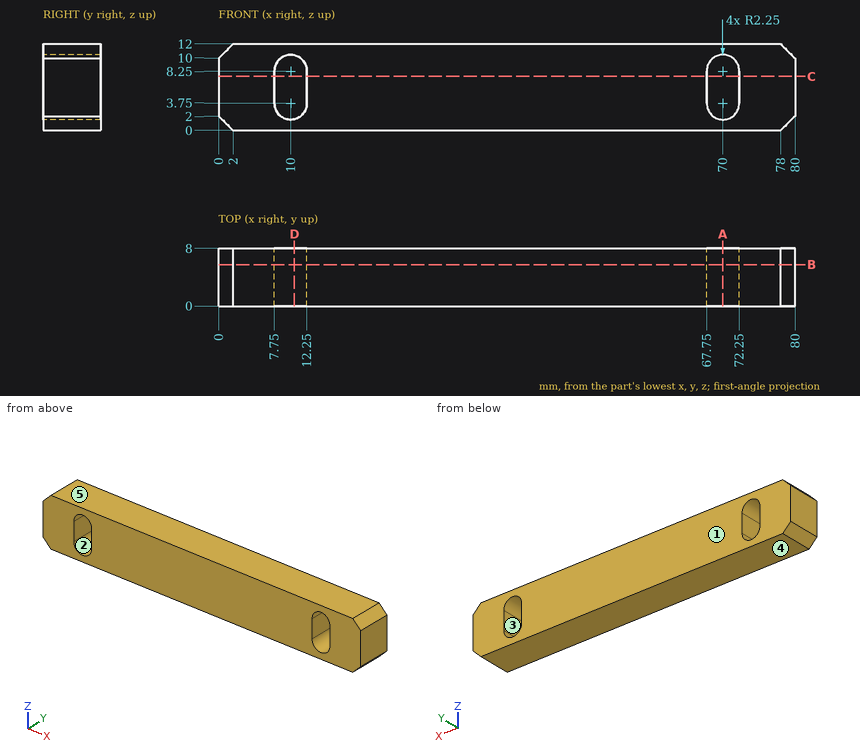
Check sheet for the drawn part. Datum: minimum x, y, z corner. Units: mm. A direction names the side the tool comes from. Round coordinates to 2 decimals unless told otherwise and drop trailing zeros. Write each loop counter-clockwise with the first axis right and the second up, starting at its lowest first coordinate (ties: lowest second). Pieces come first, ordered by that corner, then holes. Notation, with made-up numbers: (4, -15) -> (24, -15) arc R30 ccw to (24, 22) -> close; hole circle Ø8 at (21.5, 74.25). An arc over 180 degrees is marked (long way). Write each question's results on one line, items separated by ' | '. Start each with the question number.
1. Cross-section at C-C (z = 7.5). Enter the section's corners in (x, y), then the cut area to 3 significant figures.
2. Set-up check for the marked faces 1 and 2: record each of +Z, -Z, +X, -X, +Y, -Y from which the full face is reachable in a straight line by a thin tool's end or side.
3. Cross-section at D-D (x = 10.5). Enter the section's corners in (y, z).
4. Cross-section at B-B (y = 5.75). Enter the section's corners in (x, z).
5. Material ranges on probe 1 along X at (y, z) = (6.5, 6.5); probe 2 along Z at (x, y) = (69, 4.75); probe 3 along Z at (x, y) = (8.5, 6.75), recorded low to high. Write a range as from..to.
6. Cross-section at A-A (x = 70). Enter the section's corners in (y, z), then the cut area to 3 significant figures.
7. Draft check along Z on the marked faces 3, 4 and 5. Enter one of: +Z half, -Z half, draft (parallel to the pull), parting line (faces both ways), or undercut.
Solutions:
1) outline: (0, 0) -> (7.75, 0) -> (7.75, 8) -> (0, 8) -> close; (12.25, 0) -> (67.75, 0) -> (67.75, 8) -> (12.25, 8) -> close; (72.25, 0) -> (80, 0) -> (80, 8) -> (72.25, 8) -> close | area: 568 mm2
2) face 1: +Z, -Z, +X, -X, +Y | face 2: +Y, -Y
3) outline: (0, 0) -> (8, 0) -> (8, 1.56) -> (0, 1.56) -> close; (0, 10.44) -> (8, 10.44) -> (8, 12) -> (0, 12) -> close
4) outline: (0, 2) -> (2, 0) -> (78, 0) -> (80, 2) -> (80, 10) -> (78, 12) -> (2, 12) -> (0, 10) -> close; hole (7.75, 3.75) arc R2.25 ccw to (12.25, 3.75) -> (12.25, 8.25) arc R2.25 ccw to (7.75, 8.25) -> close; hole (67.75, 3.75) arc R2.25 ccw to (72.25, 3.75) -> (72.25, 8.25) arc R2.25 ccw to (67.75, 8.25) -> close
5) probe 1: x = 0..7.75, 12.25..67.75, 72.25..80 | probe 2: z = 0..1.73, 10.27..12 | probe 3: z = 0..2.07, 9.93..12
6) outline: (0, 0) -> (8, 0) -> (8, 1.5) -> (0, 1.5) -> close; (0, 10.5) -> (8, 10.5) -> (8, 12) -> (0, 12) -> close | area: 24.0 mm2
7) face 3: undercut | face 4: -Z half | face 5: +Z half
